Geometry check sheet. Reference: the model listing, model coordinates, mm. A direction names the side the tool comes from. Round coordinates to 2 decimals unless told otherwise and drop trailing zeros. Write each loop counter-clockwise with the first axis right and the second up, starting at its lowest first coordinate (ties: lowest second). Pieces come first, ordered by that corner, then holes. Notation, with made-up numbers: M 14,-15 L 45,-15 A24 ccw 45,9 Z; hole C 6,-6 d11. An arc over 180 degrees is marked long. Answer in a Markdown table with one row per item. Add a question column.
from build123d import *

# Parameters (mm, degrees)
BASE_PLATE_DEPTH           = 15
END_PAD_1_SKETCH_W         = 50
END_PAD_1_SKETCH_H         = 15
END_PAD_1_DEPTH            = 5
END_PAD_2_SKETCH_W         = 50
END_PAD_2_SKETCH_H         = 15
END_PAD_2_DEPTH            = 5
HUB_SKETCH_R               = 20
HUB_40_DEPTH               = 15
BORE_SKETCH_R              = 10
BORE_20_DEPTH              = 15
MOUNTING_HOLES_SKETCH_R    = 5
MOUNTING_HOLES_4X_10_DEPTH = 15
SIDE_NOTCH_DEPTH           = 15


with BuildPart() as part:
    # Base Plate Sketch → Base Plate (new body)
    with BuildSketch(Plane.XY):
        with BuildLine():
            Line((-10, 50), (-10, 0))
            ThreePointArc((-10, 0), (0, -10), (10, 0))
            Line((10, 0), (10, 10))
            Line((10, 10), (60, 10))
            Line((60, 10), (60, 0))
            ThreePointArc((60, 0), (70, -10), (80, 0))
            Line((80, 0), (80, 50))
            ThreePointArc((80, 50), (70, 60), (60, 50))
            Line((60, 50), (60, 40))
            Line((60, 40), (10, 40))
            Line((10, 40), (10, 50))
            ThreePointArc((10, 50), (0, 60), (-10, 50))
        make_face()
    extrude(amount=BASE_PLATE_DEPTH)

    # End Pad 1 Sketch → End Pad 1 (add)
    with BuildSketch(Plane(origin=(0, 40, 0), x_dir=(1, 0, 0), z_dir=(0, 1, 0))):
        with Locations((35, -7.5)):
            Rectangle(END_PAD_1_SKETCH_W, END_PAD_1_SKETCH_H)
    extrude(amount=END_PAD_1_DEPTH)

    # End Pad 2 Sketch → End Pad 2 (add)
    with BuildSketch(Plane.XZ.offset(-10)):
        with Locations((35, 7.5)):
            Rectangle(END_PAD_2_SKETCH_W, END_PAD_2_SKETCH_H)
    extrude(amount=END_PAD_2_DEPTH)

    # Hub Sketch → Hub Ø40 (add)
    with BuildSketch(Plane.XY.offset(15)):
        with Locations(Location((35, 25, 0), (0, 0, 270))):
            Circle(HUB_SKETCH_R)
    extrude(amount=HUB_40_DEPTH)

    # Bore Sketch → Bore Ø20 (cut)
    with BuildSketch(Plane.XY.offset(30)):
        with Locations((35, 25)):
            Circle(BORE_SKETCH_R)
    extrude(amount=-BORE_20_DEPTH, mode=Mode.SUBTRACT)

    # Mounting Holes Sketch → Mounting Holes 4xØ10 (cut)
    with BuildSketch(Plane.XY.offset(15)):
        with Locations((70, 50)):
            Circle(MOUNTING_HOLES_SKETCH_R)
        with Locations((70, 0)):
            Circle(MOUNTING_HOLES_SKETCH_R)
        Circle(MOUNTING_HOLES_SKETCH_R)
        with Locations((0, 50)):
            Circle(MOUNTING_HOLES_SKETCH_R)
    extrude(amount=-MOUNTING_HOLES_4X_10_DEPTH, mode=Mode.SUBTRACT)

    # Side Notch Sketch → Side Notch (cut)
    with BuildSketch(Plane.XY.offset(15)):
        with BuildLine():
            Line((-10, 30), (-10, 20))
            Line((-10, 20), (5, 20))
            ThreePointArc((5, 20), (10, 25), (5, 30))
            Line((5, 30), (-10, 30))
        make_face()
    extrude(amount=-SIDE_NOTCH_DEPTH, mode=Mode.SUBTRACT)


solid = part.part
Item 1: Section check D-D, the plane y = -1. Record the boundary of the cut face in (x, z), and give its area (3 significant figures).
Item 2: Gauge pin test, flat ends, axial feed: pin 1 Ø11.5 at (x, y) = (0, 0) entering from +Z; pin 2 Ø3 at (y, z) = (43, 23.5) entering from -X; pin 3 Ø9 at (x, y) = (70, 50) entering from -Z; pin 4 Ø7.5 at (x, z) = (32.5, 7) entering from +Y. Record the tip position at first contact, or that the pin passes through.
Item 3: Access from +Z, -Z, +X, -X, +Y, -Y to the whole of each face (thin tool, end or side, straight path). Record for faces 1 (the flat face through (60, 3, 7)), 2 (the cylindrical face through (74.619, -1.915, 7.605)), 3 (the flat face through (35, 45, 7)), 4 (the cylindrical face through (33.698, 34.915, 22.605)), 5 (the flat face through (-10, 10, 7)).
Item 4: Section check B-B, the plane x = 0. Record the boundary of the cut face in (y, z).
Item 5: Mould release check, pull along X, two halves, no side actions. Record for faces 6 (the cylindrical face through (54.83, 27.6, 22.4)), 7 (the cylindrical face through (-1.08, -4.88, 7.6)), 8 (the cylindrical face through (-0.651, 54.957, 7.605)), 9 (the flat face through (34, 25, 0)): +X half, -X half, draft (parallel to the pull), parting line (faces both ways), or undercut.
Item 6: Scan lines: probe 1 along Y at (x, z) = (70, 7); probe 2 along X at (y, z) = (51, 10); probe 3 along Y at (x, z) = (35, 24). Record each from-to range of solid material in increasing order. Write a range as from..to.
Item 7: Section check A-A, the plane x = 70. Record the boundary of the cut face in (y, z), and give its area (3 significant figures).
Item 8: Section check C-C, the plane z = 9. Record the boundary of the cut face in (x, y), and give its area (3 significant figures).
Result sheet:
| question | item | result |
|---|---|---|
| 1 | outline | M -9.95,0 L -4.9,0 L -4.9,15 L -9.95,15 Z; M 4.9,0 L 9.95,0 L 9.95,15 L 4.9,15 Z; M 60.05,0 L 65.1,0 L 65.1,15 L 60.05,15 Z; M 74.9,0 L 79.95,0 L 79.95,15 L 74.9,15 Z |
| 1 | area | 303 mm^2 |
| 2 | pin 1 | stops at z = 15 |
| 2 | pin 2 | stops at x = 23.7 |
| 2 | pin 3 | passes through |
| 2 | pin 4 | stops at y = 45 |
| 3 | face 1 | +Z, -Z, -Y |
| 3 | face 2 | +Z, -Z |
| 3 | face 3 | +Z, -Z, +Y |
| 3 | face 4 | +Z |
| 3 | face 5 | +Z, -Z, -X, +Y, -Y |
| 4 | outline | M -10,0 L -5,0 L -5,15 L -10,15 Z; M 5,0 L 20,0 L 20,15 L 5,15 Z; M 30,0 L 45,0 L 45,15 L 30,15 Z; M 55,0 L 60,0 L 60,15 L 55,15 Z |
| 5 | face 6 | parting line |
| 5 | face 7 | undercut |
| 5 | face 8 | undercut |
| 5 | face 9 | draft |
| 6 | probe 1 | y = -10..-5, 5..45, 55..60 |
| 6 | probe 2 | x = -9.95..-4.9, 4.9..9.95, 60.05..65.1, 74.9..79.95 |
| 6 | probe 3 | y = 5..15, 35..45 |
| 7 | outline | M -10,0 L -5,0 L -5,15 L -10,15 Z; M 5,0 L 45,0 L 45,15 L 5,15 Z; M 55,0 L 60,0 L 60,15 L 55,15 Z |
| 7 | area | 750 mm^2 |
| 8 | outline | M -10,0 A10 ccw 10,0 L 10,5 L 60,5 L 60,0 A10 ccw 80,0 L 80,50 A10 ccw 60,50 L 60,45 L 10,45 L 10,50 A10 ccw -10,50 L -10,30 L 5,30 A5 cw 5,20 L -10,20 Z; hole C 0,0 d10; hole C 0,50 d10; hole C 70,0 d10; hole C 70,50 d10 |
| 8 | area | 4,120 mm^2 |
